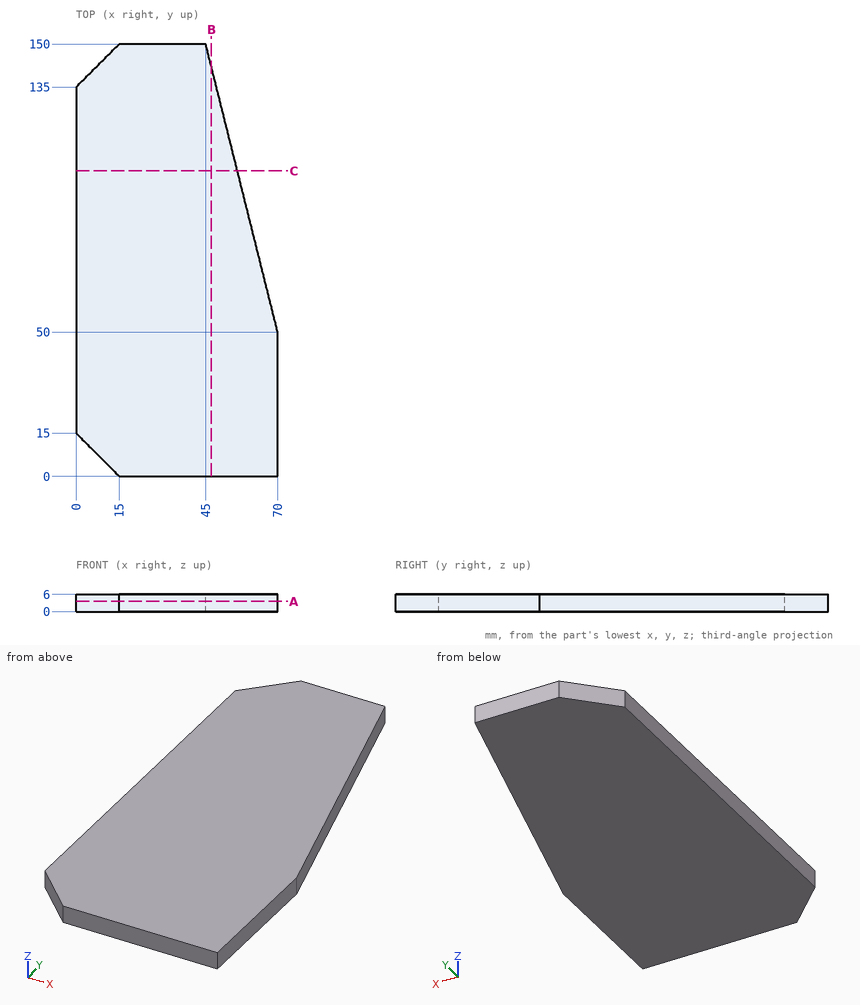
Job drawing, mm, ordinate dimensions from the low corner. One solid piece. Give positions to 0.01 mm unless a question says otherwise; leave off trailing zeros. Write each loop counter-clockwise with the first axis right and the second up, starting at its lowest first coordinate (ties: lowest second). Pieces come first, ordered by that corner, then holes. Notation, with made-up numbers: M 34.25,88 L 92.25,88 A33 cw 92.25,124 Z; hole C 31,63.5 d8. An arc over 180 degrees is marked long. One line per item, written item: value. Start each with the question number.
Q1. Probe probe 1 along X at (y, z) = (82.5, 5.1) (3 decimals); probe 2 along Y at (x, z) = (7, 4.9); probe 3 along X at (y, z) = (11, 4.15). List the from-to ranges inside material, lowest first. Write a range as [from, to].
Q2. Saw through at A-A, the plane z = 3.5. Write the cut outline in (x, y).
Q3. Saw through at B-B, the plane x = 47. Write the cut outline in (y, z).
Q4. Saw through at C-C, the plane y = 106. Write the cut outline in (x, z).
Output values:
1. probe 1: x = [0, 61.875]
1. probe 2: y = [8, 142]
1. probe 3: x = [4, 70]
2. outline: M 0,15 L 15,0 L 70,0 L 70,50 L 45,150 L 15,150 L 0,135 Z
3. outline: M 0,0 L 142,0 L 142,6 L 0,6 Z
4. outline: M 0,0 L 56,0 L 56,6 L 0,6 Z
